from build123d import *

# Parameters (mm, degrees)
BOSS_EXTRUDE1_DEPTH  = 30
SKETCH5_W            = 75
SKETCH5_H            = 130
CUT_EXTRUDE3_DEPTH   = 433.897216438
FILLET2_R            = 15
FILLET2_OF_MIRROR3_R = 15
FILLET3_R            = 30


with BuildPart() as part:
    # Sketch1 → Boss-Extrude1 (new, symmetric)
    with BuildSketch(Plane.XY):
        with BuildLine():
            Line((42.5, 0), (320, 0))
            Line((320, 0), (320, 220))
            Line((320, 220), (125, 220))
            ThreePointArc((125, 220), (110.857864376, 225.857864376), (105, 240))
            Line((105, 240), (105, 270))
            ThreePointArc((105, 270), (99.142135624, 284.142135624), (85, 290))
            Line((85, 290), (-85, 290))
            ThreePointArc((-85, 290), (-99.142135624, 284.142135624), (-105, 270))
            Line((-105, 270), (-105, 240))
            ThreePointArc((-105, 240), (-110.857864376, 225.857864376), (-125, 220))
            Line((-125, 220), (-320, 220))
            Line((-320, 220), (-320, 0))
            Line((-320, 0), (-42.5, 0))
            Line((-42.5, 0), (-42.5, 150))
            ThreePointArc((-42.5, 150), (0, 192.5), (42.5, 150))
            Line((42.5, 150), (42.5, 0))
        make_face()
        with BuildLine():
            Line((45, 220), (-45, 220))
            ThreePointArc((-45, 220), (-55.606601718, 224.393398282), (-60, 235))
            Line((-60, 235), (-60, 255))
            ThreePointArc((-60, 255), (-55.606601718, 265.606601718), (-45, 270))
            Line((-45, 270), (45, 270))
            ThreePointArc((45, 270), (55.606601718, 265.606601718), (60, 255))
            Line((60, 255), (60, 235))
            ThreePointArc((60, 235), (55.606601718, 224.393398282), (45, 220))
        make_face(mode=Mode.SUBTRACT)
    extrude(amount=BOSS_EXTRUDE1_DEPTH, both=True)

    # Sketch5 → Cut-Extrude3 (cut, symmetric)
    with BuildSketch(Plane.XY):
        with Locations((-245, 110)):
            Rectangle(SKETCH5_W, SKETCH5_H)
        with Locations((-125, 110)):
            Rectangle(SKETCH5_W, SKETCH5_H)
    cut_extrude3 = extrude(amount=CUT_EXTRUDE3_DEPTH, both=True, mode=Mode.SUBTRACT)

    # Fillet2
    fillet2_edges = [part.edges().sort_by_distance(p)[0] for p in [
        (-207.5, 175, 0),
        (-207.5, 45, 0),
        (-282.5, 45, 0),
        (-282.5, 175, 0),
        (-87.5, 175, 0),
        (-87.5, 45, 0),
        (-162.5, 45, 0),
        (-162.5, 175, 0),
    ]]
    fillet(fillet2_edges, radius=FILLET2_R)

    # Mirror3: Cut-Extrude3 across plane
    add(cut_extrude3.mirror(Plane(origin=(0, 0, 0), x_dir=(0, 0, 1), z_dir=(1, 0, 0))), mode=Mode.SUBTRACT)

    # Fillet2 of Mirror3
    fillet2_of_mirror3_edges = [part.edges().sort_by_distance(p)[0] for p in [
        (207.5, 175, 0),
        (207.5, 45, 0),
        (282.5, 45, 0),
        (282.5, 175, 0),
        (87.5, 175, 0),
        (87.5, 45, 0),
        (162.5, 45, 0),
        (162.5, 175, 0),
    ]]
    fillet(fillet2_of_mirror3_edges, radius=FILLET2_OF_MIRROR3_R)

    # Fillet3
    fillet3_edges = [part.edges().sort_by_distance(p)[0] for p in [
        (-42.5, 0, 0),
        (-320, 0, 0),
        (-320, 220, 0),
        (320, 220, 0),
        (320, 0, 0),
        (42.5, 0, 0),
    ]]
    fillet(fillet3_edges, radius=FILLET3_R)


solid = part.part
Check sheet for the modelled part. Datum: model origin and axes. Units: mm. A direction names the side the tool comes from. Give positions to 0.01 mm unless a question says otherwise; leave off trailing zeros. Write each loop counter-clockwise with the first axis right and the second up, starting at its lowest first coordinate (ties: lowest second). Pieces come first, ordered by that corner, then holes. Notation, with made-up numbers: (78, 59) -> (106, 59) arc R25 ccw to (106, 76) -> close; hole circle Ø6 at (67, -35.75). An arc over 180 degrees is marked (long way). Use one line per item in the form item = value. Start each with the question number.
1. Go/stop test with flat-tipped pins: P1, Ø16, axis at y = 249.5, z = -10.5, coming from the -X side; P2, Ø22.5, axis at x = -119.5, z = 12.5, coming from the +Y side; P3, Ø22.5, axis at x = 135.5, z = 2, coming from the +Y side. Record where each tip stops, or that it passes through.
2. Section check B-B (y = 122). Record the cut outline in (x, z), and give its area (3 significant figures).
3. Section check D-D (z = -15.5). Count the separate pieces of the cut face and the enclosed holes in it, and give its area (3 significant figures).
4. Section check A-A (x = 0). Record the cut outline in (y, z), and give its area (3 significant figures).
5. Thickness scan on line 1 along X through (y, z) = (95.5, -6); line 2 along X through (y, z) = (43, -19.5); line 3 along Y through (x, z) = (-230.5, 16). Record the ranges inside material, lowest first. Write a range as from..to.
6. Mould release check, pull along Y, two halves, no side actions. Record for faces 1 (the flat face through (105, 255, 0)), 2 (the cylindrical face through (311.445, 210.979, 0.42)), 3 (the flat face through (-1, 270, 0)): pulls with the +Y half, pulls with the -Y half, needs draft (parallel to the pull), parting line crosses it, or undercut.
7. Access from +Z, -Z, +X, -X, +Y, -Y to the whole of each face (thin tool, end or side, straight path). Record for faces 4 (the cylindrical face through (-51.055, 9.021, -0.42)), 5 (the flat face through (180, 0, 0)), 6 (the flat face through (-125, 45, 0)).
8. Section check C-C (y = 37). Record the cut outline in (x, z).
Conclusion:
q1.P1 = -105
q1.P2 = 229.07
q1.P3 = 220.01
q2.outline = (-320, -30) -> (-282.5, -30) -> (-282.5, 30) -> (-320, 30) -> close; (-207.5, -30) -> (-162.5, -30) -> (-162.5, 30) -> (-207.5, 30) -> close; (-87.5, -30) -> (-42.5, -30) -> (-42.5, 30) -> (-87.5, 30) -> close; (42.5, -30) -> (87.5, -30) -> (87.5, 30) -> (42.5, 30) -> close; (162.5, -30) -> (207.5, -30) -> (207.5, 30) -> (162.5, 30) -> close; (282.5, -30) -> (320, -30) -> (320, 30) -> (282.5, 30) -> close
q2.area = 15,300 mm²
q3.separate_pieces = 1
q3.enclosed_holes = 5
q3.area = 94,700 mm²
q4.outline = (192.5, -30) -> (220, -30) -> (220, 30) -> (192.5, 30) -> close; (270, -30) -> (290, -30) -> (290, 30) -> (270, 30) -> close
q4.area = 2,850 mm²
q5.line_1 = -320..-282.5, -207.5..-162.5, -87.5..-42.5, 42.5..87.5, 162.5..207.5, 282.5..320
q5.line_2 = -320..-42.5, 42.5..320
q5.line_3 = 0..45, 175..220
q6.face_1 = needs draft
q6.face_2 = pulls with the +Y half
q6.face_3 = undercut
q7.face_4 = +Z, -Z, -Y
q7.face_5 = +Z, -Z, +X, -X, -Y
q7.face_6 = +Z, -Z
q8.outline = (-320, -30) -> (-42.5, -30) -> (-42.5, 30) -> (-320, 30) -> close; (42.5, -30) -> (320, -30) -> (320, 30) -> (42.5, 30) -> close
